For this review, use the dimensioned drawing (mm, ordinates from the lowest corner) and the shaded views. Coordinates: 2 decimals unless noted, no trailing zeros. Loops run counter-clockwise (first coordinate to the right, second up) from the corner with the lowest first, then second, coordinate; pieces in that order, holes last. Notation, with made-up numbers: (-21, 67.5) - (-9, 67.5) arc R13 ccw to (-9, 71.5) - close; hole circle Ø7 at (-6, -0.5). An arc over 180 degrees is marked (long way). Answer in a Markdown table with one row per item. Add a question column.
(1) We need section A-A on y = 6.5. Write out the cut boundary in (x, z) (1 decimal), plus the area to 3 significant figures.
(2) For line 1 along Z through (x, y) = (14.5, 3); line 2 along Z through (x, y) = (17, 4); line 3 along X through (y, z) = (6.25, 16.75) (1 decimal), list the stretches that pass through material, from the lowest coordinate up.
(3) For P1, Ø1.5, axis at y = 3, z = 18.5, coming from the +X side; P2, Ø1, axis at y = 4.5, z = 8, coming from the -X side, all flat-tipped, find the tip position at first contact; note any pin that passes through.
(4) Mouldability with a two-part tool opening along Z and no side actions: class the marked faces 1, 2 and 3 as +Z half, -Z half, draft (parallel to the pull), parting line (faces both ways), or undercut.
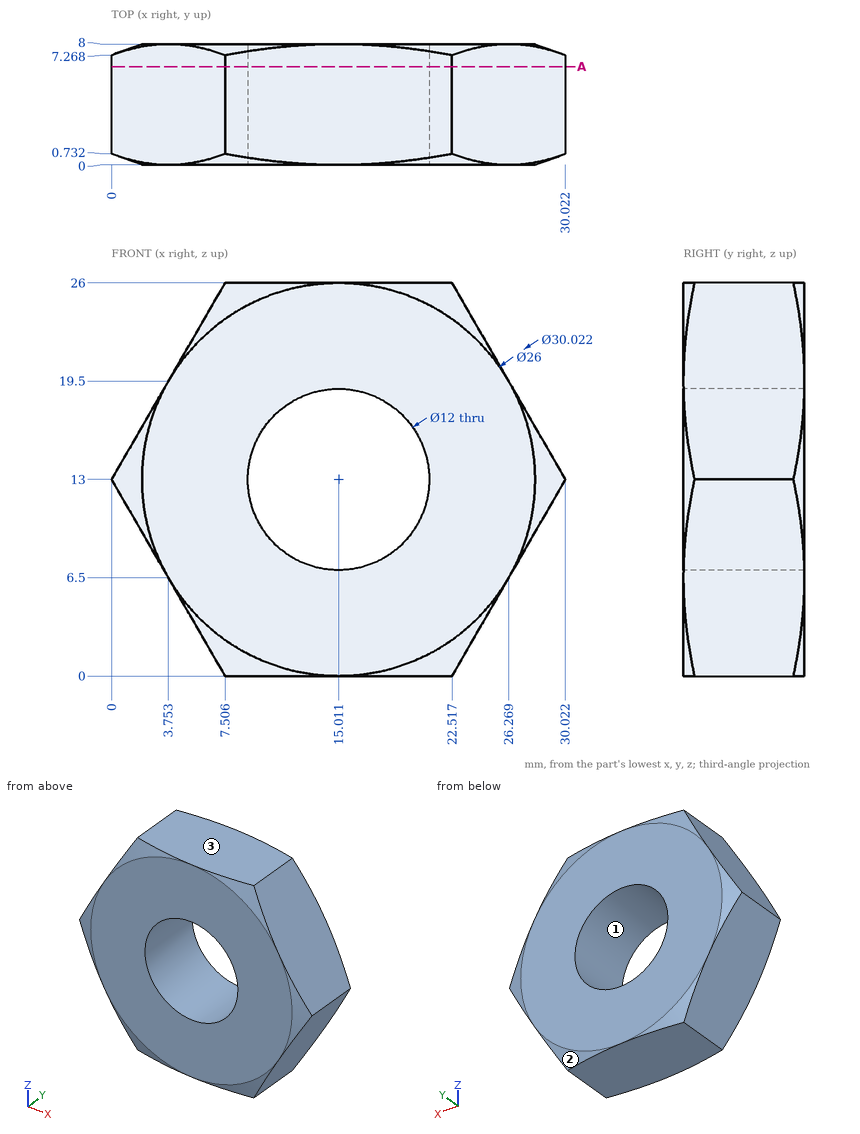
Outcome:
| question | item | result |
|---|---|---|
| 1 | outline | (0, 13) - (7.5, 0) - (22.5, 0) - (30, 13) - (22.5, 26) - (7.5, 26) - close; hole circle Ø12 at (15, 13) |
| 1 | area | 472 mm² |
| 2 | line 1 | 0 to 7.02, 18.98 to 26 |
| 2 | line 2 | 0 to 7.34, 18.66 to 26 |
| 2 | line 3 | 2.2 to 10.3, 19.7 to 27.9 |
| 3 | P1 | x = 27.28 |
| 3 | P2 | x = 2.6 |
| 4 | face 1 | undercut |
| 4 | face 2 | -Z half |
| 4 | face 3 | +Z half |
